Build history of the part. All positions in model axes, mm. A direction names the side the tool comes from. Round coordinates to 2 decimals unless told otherwise and drop trailing zeros. Loops run counter-clockwise (first coordinate to the right, second up) from the corner with the lowest first, then second, coordinate; pieces in that order, holes last. Notation, with made-up numbers: M -26,-9 L -17,-9 A27 ccw -17,27 Z; hole C 13.5,27 d5. An arc over 180 degrees is marked long. Write each question's results on one line, items separated by ' | '. Start each with the question number.
```python
from build123d import *

# Parameters (mm, degrees)
SKETCH1_W          = 30
SKETCH1_H          = 20
CHAMFER1_SIZE      = 3
SKETCH2_W          = 18
SKETCH2_H          = 16
CUT_EXTRUDE1_DEPTH = 38
CIRPATTERN1_COUNT  = 6


with BuildPart() as part:
    # Sketch1 → Revolve1 (revolve)
    with BuildSketch(Plane(origin=(0, 0, 0), x_dir=(0, 0, -1), z_dir=(1, 0, 0)), mode=Mode.PRIVATE) as revolve1_sk:
        with Locations((15, 125)):
            Rectangle(SKETCH1_W, SKETCH1_H)
    revolve(revolve1_sk.sketch.rotate(Axis((0, 0, 0), (0, 0, -1)), 90), axis=Axis((0, 0, 0), (0, 0, -1)))

    # Chamfer1
    chamfer1_edges = [part.edges().sort_by_distance(p)[0] for p in [
        (-135, 0, -30),
        (-135, 0, 0),
    ]]
    chamfer(chamfer1_edges, length=CHAMFER1_SIZE)

    # Sketch2 → Cut-Extrude1 (cut)
    with BuildSketch(Plane.XY):
        with Locations((0, 135)):
            Rectangle(SKETCH2_W, SKETCH2_H)
    cut_extrude1 = extrude(amount=-CUT_EXTRUDE1_DEPTH, mode=Mode.SUBTRACT)

    # CirPattern1: Cut-Extrude1 ×6 about axis
    cirpattern1_axis = Axis((0, 0, 0), (0, 0, 1))
    for i in range(1, CIRPATTERN1_COUNT):
        add(cut_extrude1.rotate(cirpattern1_axis, i * 360 / CIRPATTERN1_COUNT), mode=Mode.SUBTRACT)


solid = part.part
```
Item 1: Drill centre lines: line 1 along Y through (x, z) = (0, -9); line 2 along X through (y, z) = (-63.5, -13); line 3 along Y through (x, z) = (60, -10). Where is each one in solid material? Low to high. Write a range as [from, to].
Item 2: Tool access for faces 5 (the flat face through (-108.77, -73.19, -14.79)), 6 (the flat face through (-117.77, 57.6, -14.79)), 7 (the flat face through (-117.77, -57.6, -14.79)), 8 (the cylindrical face through (134.997, 0.864, -15.168)): list every direction of +Z, -Z, +X, -X, +Y, -Y with a clear straight run to the whole face (end or side of a thin tool).
Item 3: Drop flat-ended pins along their axis: pin 1 (4 mm diameter, centred on x = 22.5, z = -6.5, fed in from -Y); pin 2 (8 mm diameter, centred on x = 28.5, z = -25, fed in from -Y); pin 3 (3 mm diameter, centred on x = 92.5, z = -27, fed in from -Y). Give the stop position or say it passes through.
Item 4: Saw through at B-B, the plane x = 0. Give the cut face in (y, z).
Item 5: Saw through at D-D, the plane y = 68. Give the cut face in (x, z), then the cut area to 3 significant figures.
Item 6: Saw through at A-A, the plane z = -11.5. Give the cut face in (x, y).
Item 7: Mould opens along Y. For faces 1 (the cylindrical face through (-68.246, 116.479, -15.168)), 2 (the flat face through (110.05, -63.39, -14.79)), 3 (the conical face through (-65.36, -114.9, -29.81)), 4 (the flat face through (108.77, -73.19, -14.79)) say: released by +Y, released by -Y, zero draft, split by the parting line, or undercut.
Item 8: Saw through at C-C, the plane y = 0. Give the cut face in (x, z).
Working result:
1) line 1: y = [-127, -115], [115, 127] | line 2: x = [-109.99, -95.88], [95.88, 109.99] | line 3: y = [-120.93, -98.11], [98.11, 120.93]
2) face 5: +Z, -Z, -X | face 6: +Z, -Z, +Y | face 7: +Z, -Z, -Y | face 8: +Z, -Z, +X
3) pin 1: stops at y = -133.43 | pin 2: stops at y = -132.76 | pin 3: stops at y = -99.72
4) outline: M -127,-30 L -115,-30 L -115,0 L -127,0 Z; M 115,-30 L 127,-30 L 127,0 L 115,0 Z
5) outline: M -107.39,-30 L -92.74,-30 L -92.74,0 L -107.39,0 Z; M 92.74,-30 L 107.39,-30 L 107.39,0 L 92.74,0 Z | area: 879 mm²
6) outline: M -121.15,-59.56 L -114.49,-55.71 L -105.49,-71.29 L -112.15,-75.14 A135 ccw -9,-134.7 L -9,-127 L 9,-127 L 9,-134.7 A135 ccw 112.15,-75.14 L 105.49,-71.29 L 114.49,-55.71 L 121.15,-59.56 A135 ccw 121.15,59.56 L 114.49,55.71 L 105.49,71.29 L 112.15,75.14 A135 ccw 9,134.7 L 9,127 L -9,127 L -9,134.7 A135 ccw -112.15,75.14 L -105.49,71.29 L -114.49,55.71 L -121.15,59.56 A135 ccw Z; hole C 0,0 d230
7) face 1: released by +Y | face 2: undercut | face 3: released by -Y | face 4: undercut
8) outline: M -135,-27 L -132,-30 L -115,-30 L -115,0 L -132,0 L -135,-3 Z; M 115,-30 L 132,-30 L 135,-27 L 135,-3 L 132,0 L 115,0 Z
